CAD build for the part. Positions are in the model's coordinates, mm. Round coordinates to 2 decimals unless told otherwise and drop trailing zeros. Loops run counter-clockwise (first coordinate to the right, second up) from the corner with the lowest first, then second, coordinate; pieces in that order, holes last.
```python
from build123d import *

# Parameters (mm, degrees)
SKETCH1_R           = 40
BOSS_EXTRUDE1_DEPTH = 16
CUT_EXTRUDE1_DEPTH  = 398.241740002


with BuildPart() as part:
    # Sketch1 → Boss-Extrude1 (new body)
    with BuildSketch(Plane.XY):
        with BuildLine():
            Line((0, 0), (39.808164115, 0))
            ThreePointArc((39.808164115, 0), (79, 48), (118.191835885, 0))
            Line((118.191835885, 0), (214.808164115, 0))
            ThreePointArc((214.808164115, 0), (254, 48), (293.191835885, 0))
            Line((293.191835885, 0), (333, 0))
            Line((333, 0), (333, 216))
            Line((333, 216), (293.191835885, 216))
            ThreePointArc((293.191835885, 216), (254, 168), (214.808164115, 216))
            Line((214.808164115, 216), (118.191835885, 216))
            ThreePointArc((118.191835885, 216), (79, 168), (39.808164115, 216))
            Line((39.808164115, 216), (0, 216))
            Line((0, 216), (0, 0))
        make_face()
        with Locations((166.5, 108)):
            Circle(SKETCH1_R, mode=Mode.SUBTRACT)
    extrude(amount=BOSS_EXTRUDE1_DEPTH)

    # Sketch2 → Cut-Extrude1 (cut, through all)
    with BuildSketch(Plane.XZ):
        Polygon((0, 16), (10.7, 0), (0, 0), align=None)
        Polygon((333, 16), (313.3, 0), (333, 0), align=None)
    extrude(amount=-CUT_EXTRUDE1_DEPTH, mode=Mode.SUBTRACT)


solid = part.part
```
Item 1: Cut at A-A, the plane y = 208. Give the cut face in (x, z), plus the area to 3 significant figures.
Answers follow:
outline: (0, 16) - (10.7, 0) - (39, 0) - (39, 16) - close; (119, 0) - (214, 0) - (214, 16) - (119, 16) - close; (294, 0) - (313.3, 0) - (333, 16) - (294, 16) - close
area: 2,520 mm2
Item 2: Flat gauge pins, fed straight in: P1, Ø1, axis at x = 40, y = 53.5, coming from the -Z side; P2, Ø2, axis at x = 82, z = 5, coming from the -Y side; P3, Ø8, axis at y = 137.5, z = 9.5, coming from the +X side. Where does each tip first touch, or does it go through?
Answers follow:
P1: stops at z = 0
P2: stops at y = 47.8
P3: stops at x = 329.92
Item 3: Cut at C-C, the plane z = 3.75. Give the cut face in (x, y).
Answers follow:
outline: (8.19, 0) - (39.81, 0) arc R40 cw (long way) to (118.19, 0) - (214.81, 0) arc R40 cw (long way) to (293.19, 0) - (317.92, 0) - (317.92, 216) - (293.19, 216) arc R40 cw (long way) to (214.81, 216) - (118.19, 216) arc R40 cw (long way) to (39.81, 216) - (8.19, 216) - close; hole circle Ø80 at (166.5, 108)
Item 4: Two-plate mould, pull along Y, no slides. Class faces 1 (the flat face through (166, 0, 8)), 2 (the flat face through (5.275, 106.488, 8.112)), 3 (the cylindrical face through (79.992, 168.012, 7.888)), 4 (the cylindrical face through (78.008, 47.988, 7.888)): released by +Y, released by -Y, zero draft, split by the parting line, or undercut.
Answers follow:
face 1: released by -Y
face 2: zero draft
face 3: undercut
face 4: undercut
Item 5: Cut at B-B, the plane y = 108. Give the cut face in (x, z).
Answers follow:
outline: (0, 16) - (10.7, 0) - (126.5, 0) - (126.5, 16) - close; (206.5, 0) - (313.3, 0) - (333, 16) - (206.5, 16) - close
Item 6: Probe line 1 (Y direction, x = 166.5, z = 3.75); line 2 (X direction, y = 44, z = 12.25); line 3 (X direction, y = 8, z = 8.25). List the from-to ranges inside material, lowest first.
Answers follow:
line 1: y = 0 to 68, 148 to 216
line 2: x = 2.51 to 61.56, 96.44 to 236.56, 271.44 to 328.38
line 3: x = 5.18 to 39, 119 to 214, 294 to 323.46
Item 7: Cut at D-D, the plane x = 176. Give the cut face in (y, z), plus the area to 3 significant figures.
Answers follow:
outline: (0, 0) - (69.14, 0) - (69.14, 16) - (0, 16) - close; (146.86, 0) - (216, 0) - (216, 16) - (146.86, 16) - close
area: 2,210 mm2
